Could you check a few things on this model? Use its own coordinates, in mm. A direction names the side the tool comes from. Round coordinates to 2 decimals unless told otherwise and drop trailing zeros. Order: outer loops, then holes, each group sorted by start corner. A loop starts at its lowest first (then second) coordinate and runs counter-clockwise, first axis right, second up. Notation, with made-up numbers: (89.5, 75) - (142.5, 75) arc R29 ccw to (142.5, 111) - close; hole circle Ø8 at (3.25, 54). An arc over 180 degrees is marked (long way). Use one line per item in the form item = value.
from build123d import *

# Parameters (mm, degrees)
SKETCH_1_W          = 50
SKETCH_1_H          = 58
EXTRUDE_1_DEPTH     = 2.8
SKETCH_2_R          = 1.65
CUT_EXTRUDE_1_DEPTH = 54.537707789
SKETCH_3_W          = 0.45
SKETCH_3_H          = 0.45
CUT_EXTRUDE_2_DEPTH = 63.005437899
CUT_EXTRUDE_3_DEPTH = 48


with BuildPart() as part:
    # 草图1 → 凸台-拉伸1 (new body)
    with BuildSketch(Plane.XY):
        with Locations((-14.007843137, -7.562745098)):
            Rectangle(SKETCH_1_W, SKETCH_1_H)
    extrude(amount=EXTRUDE_1_DEPTH)

    # 草图2 → 切除-拉伸1 (cut, through all)
    with BuildSketch(Plane.XY.offset(2.8)):
        with Locations((-29.007843137, 18.937254902)):
            Circle(SKETCH_2_R)
        with Locations((-35.007843137, 2.437254902)):
            Circle(SKETCH_2_R)
        with Locations((-25.007843137, 2.437254902)):
            Circle(SKETCH_2_R)
        with Locations((5.992156863, 2.437254902)):
            Circle(SKETCH_2_R)
        with Locations((-35.007843137, -17.562745098)):
            Circle(SKETCH_2_R)
        with Locations((-25.007843137, -17.562745098)):
            Circle(SKETCH_2_R)
        with Locations((-29.007843137, -34.062745098)):
            Circle(SKETCH_2_R)
        with Locations((5.992156863, -17.562745098)):
            Circle(SKETCH_2_R)
    extrude(amount=-CUT_EXTRUDE_1_DEPTH, mode=Mode.SUBTRACT)

    # 草图3 → 切除-拉伸2 (cut, through all)
    with BuildSketch(Plane(origin=(10.992156863, 0, 0), x_dir=(0, 0, -1), z_dir=(1, 0, 0))):
        with Locations((-0.225, -8.587745098)):
            Rectangle(SKETCH_3_W, SKETCH_3_H)
    extrude(amount=-CUT_EXTRUDE_2_DEPTH, mode=Mode.SUBTRACT)

    # 草图5 → 切除-拉伸3 (cut)
    with BuildSketch(Plane(origin=(0, 16.437254902, 0), x_dir=(1, 0, 0), z_dir=(0, 1, 0))):
        with BuildLine():
            Line((-2.794148584, -2.8), (-15.22153769, -2.8))
            ThreePointArc((-15.22153769, -2.8), (-13.675866521, -1.129773625), (-11.700425541, 0))
            Line((-11.700425541, 0), (-6.408228111, 0.035055203))
            ThreePointArc((-6.408228111, 0.035055203), (-4.378805339, -1.098982371), (-2.794148584, -2.8))
        make_face()
    extrude(amount=-CUT_EXTRUDE_3_DEPTH, mode=Mode.SUBTRACT)


solid = part.part
Item 1: I need wall thicknesses on L1, parallel to Y at x = -4.5, z = 0.35; L2, parallel to Y at x = 6.5, z = 2.2; L3, parallel to X at y = -18, z = 0.7. Which ranges of each line are inside material? Lowest first, please.
Found:
L1 = -36.56 to -8.81, -8.36 to 21.44
L2 = -36.56 to -19.13, -15.99 to 0.87, 4.01 to 21.44
L3 = -39.01 to -36.6, -33.42 to -26.6, -23.42 to -13.08, -4.94 to 4.4, 7.58 to 10.99
Item 2: Imagine slicing it at A-A on x = -8.5. Please give me the cut outline in (y, z), plus the area to 3 significant figures.
Found:
outline = (-36.56, 0) - (-31.56, 0) - (-31.56, 2.8) - (-36.56, 2.8) - close; (16.44, 0) - (21.44, 0) - (21.44, 2.8) - (16.44, 2.8) - close
area = 28.0 mm2
Item 3: For faces 4 (the face through (-4.365, -7.227, 1.11)), 5 (the face through (10.992, -8, 1)), which set-ups out of +Z, -Z, +X, -X, +Y, -Y let a thin tool reach every point of the face, with its end or its side?
Found:
face_4 = +Z
face_5 = +Z, -Z, +X, +Y, -Y
Item 4: If we mould it in two halves opening along X, with no side actions, what happens to faces 1 (the face through (-14, 7, 0)), 2 (the face through (-39.008, -8, 1)), 3 (the face through (5.777, -15.927, 1.42))? For each: released by +X, released by -X, zero draft, split by the parting line, or undercut.
Found:
face_1 = zero draft
face_2 = released by -X
face_3 = undercut
Item 5: Imagine slicing it at C-C on z = 1.15. State how many separate pieces and enclosed holes the cut face has, plus the area to 3 significant figures.
Found:
separate_pieces = 1
enclosed_holes = 9
area = 2,380 mm2
Item 6: Imagine slicing it at D-D on x = 5.5. Please give me the cut outline in (y, z).
Found:
outline = (-36.56, 0) - (-19.14, 0) - (-19.14, 2.8) - (-36.56, 2.8) - close; (-15.99, 0) - (-8.81, 0) - (-8.81, 0.45) - (-8.36, 0.45) - (-8.36, 0) - (0.86, 0) - (0.86, 2.8) - (-15.99, 2.8) - close; (4.01, 0) - (21.44, 0) - (21.44, 2.8) - (4.01, 2.8) - close
Item 7: Imagine slicing it at B-B on y = -22.5. Please give me the cut outline in (x, z), plus the area to 3 significant figures.
Found:
outline = (-39.01, 0) - (-11.7, 0) arc R7.5 cw to (-15.22, 2.8) - (-39.01, 2.8) - close; (-6.32, 0) - (10.99, 0) - (10.99, 2.8) - (-2.79, 2.8) arc R7.5 cw to start
area = 113 mm2
